Model file for the job. Use its own axes, mm. Face numbers are marked on the shaded views. Round coordinates to 2 decimals unless told otherwise and drop trailing zeros. Loops run counter-clockwise (first coordinate to the right, second up) from the corner with the lowest first, then second, coordinate; pieces in that order, holes last. Notation, with made-up numbers: M 69.25,68 L 84.25,68 A19 cw 84.25,101 Z; hole C 0,-21.5 d6. An arc over 180 degrees is marked long. Use a Markdown table: item, result. Add a question column.
Item 1: Pin check, flat tips, straight feed: P1, Ø7, axis at x = -26.6, y = -55.61, coming from the +Z side; P2, Ø2, axis at x = -27.5, y = -63.5, coming from the -Z side. Stop position of each tip, or through.
Item 2: Saw through at C-C on z = 3.65. Write the cut outline in (x, y), then the cut area to 3 significant figures.
Item 3: Two-plate mould, pull along X, no slides. Class the marked faces 1, 2 and 3: +X half, -X half, draft (parallel to the pull), parting line (faces both ways), or undercut.
Item 4: Wall check: L1, parallel to Y at x = -26.6, z = 3.1; L2, parallel to X at y = -58.25, z = 4.7; L3, parallel to X at y = -54.75, z = 4.05. Give the ranges that are in metal, low to high. Write a range as from..to.
Item 5: Saw through at B-B on y = -59.5. Write the cut outline in (x, z), then the cut area to 3 significant figures.
Item 6: Saw through at A-A on x = -26.6. Write the cut outline in (y, z).
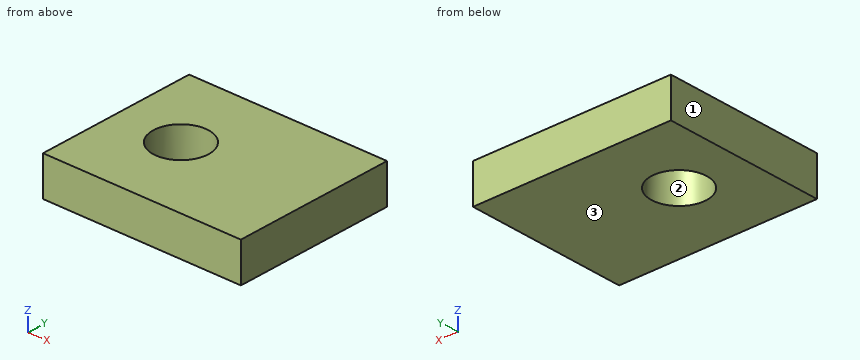
```python
from build123d import *

# Parameters (mm, degrees)
SKETCH1_W           = 30.5
SKETCH1_H           = 25
SKETCH1_R           = 4.25
BOSS_EXTRUDE1_DEPTH = 6


with BuildPart() as part:
    # Sketch1 → Boss-Extrude1 (new body)
    with BuildSketch(Plane.XY):
        with Locations((-21.35, -55.605666667)):
            Rectangle(SKETCH1_W, SKETCH1_H)
        with Locations((-26.6, -55.605666667)):
            Circle(SKETCH1_R, mode=Mode.SUBTRACT)
    extrude(amount=BOSS_EXTRUDE1_DEPTH)


solid = part.part
```
Entries:
| question | item | result |
|---|---|---|
| 1 | P1 | through |
| 1 | P2 | z = 0 |
| 2 | outline | M -36.6,-68.11 L -6.1,-68.11 L -6.1,-43.11 L -36.6,-43.11 Z; hole C -26.6,-55.61 d8.5 |
| 2 | area | 706 mm2 |
| 3 | face 1 | -X half |
| 3 | face 2 | undercut |
| 3 | face 3 | draft |
| 4 | L1 | -68.11..-59.86, -51.36..-43.11 |
| 4 | L2 | -36.6..-29.93, -23.27..-6.1 |
| 4 | L3 | -36.6..-30.76, -22.44..-6.1 |
| 5 | outline | M -36.6,0 L -28.3,0 L -28.3,6 L -36.6,6 Z; M -24.9,0 L -6.1,0 L -6.1,6 L -24.9,6 Z |
| 5 | area | 163 mm2 |
| 6 | outline | M -68.11,0 L -59.86,0 L -59.86,6 L -68.11,6 Z; M -51.36,0 L -43.11,0 L -43.11,6 L -51.36,6 Z |
